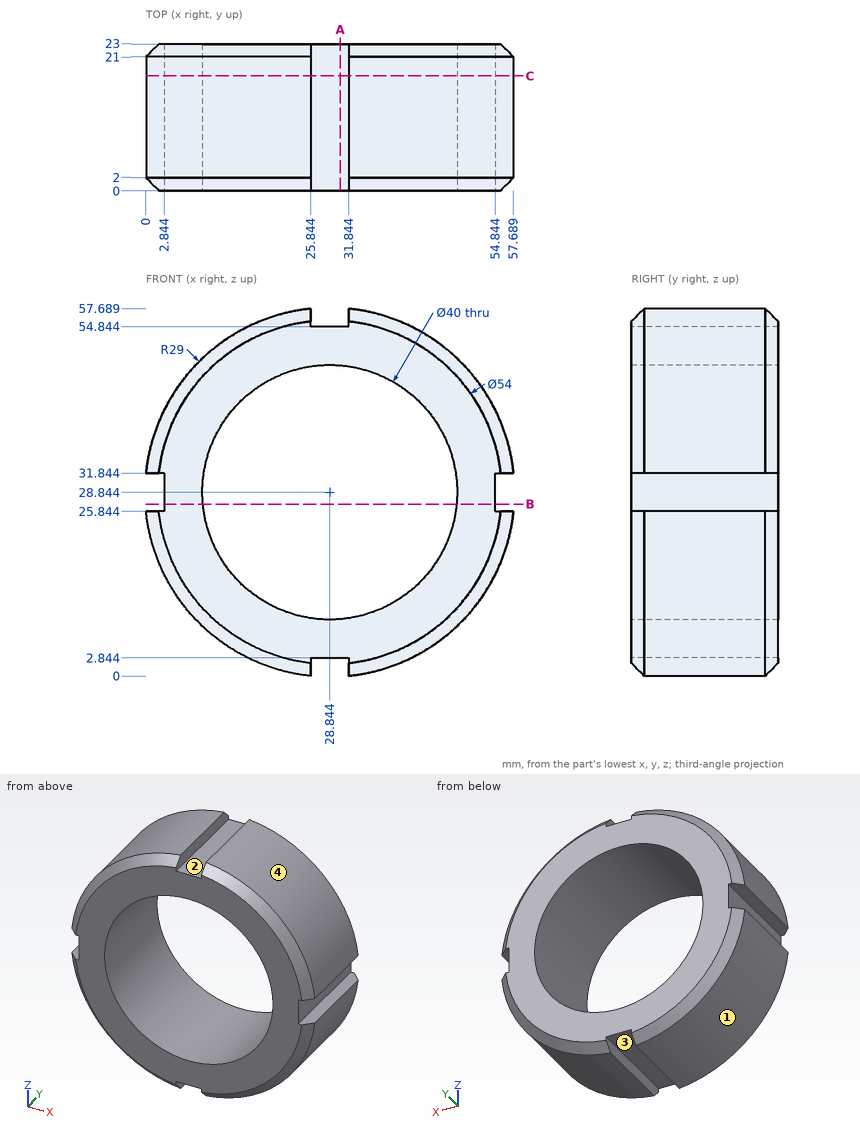
Can you work these out from the drawing? Everything is in mm from the part's minimum corner. Coordinates: 2 decimals unless noted, no trailing zeros. Loops run counter-clockwise (first coordinate to the right, second up) from the corner with the lowest first, then second, coordinate; pieces in that order, holes last.
1. For P1, Ø2.5, axis at x = 56.5, y = 10, coming from the +Z side (1 decimal); P2, Ø1.8, axis at x = 28.5, y = 14, coming from the +Z side; P3, Ø10, axis at y = 8, z = 38, coming from the -X side, each with a flat end and sliding along its axis, tell me the tip position at first contact or that it passes through.
2. I need wall thicknesses on L1, parallel to Z at x = 29, y = 14 (1 decimal); L2, parallel to Z at x = 26, y = 9.75 (1 decimal); L3, parallel to X at y = 9.5, z = 25. Which ranges of each line are inside material? Lowest first, please.
3. Imagine slicing it at C-C, the plane y = 18. Please give me the cut outline in (x, z) (1 decimal).
4. Imagine slicing it at A-A, the plane x = 30.5. Please give me the cut outline in (y, z) (1 decimal), and give its area (3 significant figures).
5. If we mould it in two halves opening along X, with no side actions, what happens to the marked faces 1, 2, 3 and 4? For each: pulls with the +X half, pulls with the -X half, needs draft (parallel to the pull), parting line crosses it, or undercut.
6. Imagine slicing it at B-B, the plane z = 27. Please give me the cut outline in (x, y) (1 decimal), and give its area (3 significant figures).
Taken from the geometry:
1. P1: stops at z = 40.8
1. P2: stops at z = 54.84
1. P3: stops at x = 0.14
2. L1: z = 2.8 to 8.8, 48.8 to 54.8
2. L2: z = 2.8 to 9, 48.6 to 54.8
2. L3: x = 0.1 to 9.22, 48.47 to 57.59
3. outline: (0, 25.8) arc R29 ccw to (25.8, 0) - (25.8, 2.8) - (31.8, 2.8) - (31.8, 0) arc R29 ccw to (57.7, 25.8) - (54.8, 25.8) - (54.8, 31.8) - (57.7, 31.8) arc R29 ccw to (31.8, 57.7) - (31.8, 54.8) - (25.8, 54.8) - (25.8, 57.7) arc R29 ccw to (0, 31.8) - (2.8, 31.8) - (2.8, 25.8) - close; hole circle Ø40 at (28.8, 28.8)
4. outline: (0, 2.8) - (23, 2.8) - (23, 8.9) - (0, 8.9) - close; (0, 48.8) - (23, 48.8) - (23, 54.8) - (0, 54.8) - close
4. area: 279 mm2
5. face 1: pulls with the -X half
5. face 2: undercut
5. face 3: undercut
5. face 4: pulls with the +X half
6. outline: (2.8, 0) - (8.9, 0) - (8.9, 23) - (2.8, 23) - close; (48.8, 0) - (54.8, 0) - (54.8, 23) - (48.8, 23) - close
6. area: 280 mm2
